```python
from build123d import *

# Parameters (mm, degrees)
CAP_BODY_DEPTH               = 23
BOLT_HOLES_12_D              = 12
SKETCH7_W                    = 17
SKETCH7_H                    = 36
HOLE_34_AT_2_COUNT           = 2
HOLE_34_AT_2_PITCH           = 78
LUBE_COUNTERBORE_SKETCH_8_R  = 4
LUBE_COUNTERBORE_8_DEPTH     = 16
LUBE_HOLE_SKETCH_6_R         = 3
LUBE_HOLE_6_DEPTH            = 72.028163461
SIDE_RELIEF_SKETCH_OUTSIDE_W = 134.804
SIDE_RELIEF_SKETCH_OUTSIDE_H = 72.804
SIDE_RELIEF_CUT_DEPTH        = 66.03076203


with BuildPart() as part:
    # Cap Profile Sketch → Cap Body (new, symmetric)
    with BuildSketch(Plane.XY):
        with BuildLine():
            Line((-22.627416998, 8), (-27.627416998, 8))
            Line((-27.627416998, 8), (-27.627416998, 24))
            Line((-27.627416998, 24), (-54, 24))
            Line((-54, 24), (-54, 36))
            Line((-54, 36), (-31.749015733, 36))
            ThreePointArc((-31.749015733, 36), (0, 48), (31.749015733, 36))
            Line((31.749015733, 36), (54, 36))
            Line((54, 36), (54, 24))
            Line((54, 24), (27.627416998, 24))
            Line((27.627416998, 24), (27.627416998, 8))
            Line((27.627416998, 8), (22.627416998, 8))
            ThreePointArc((22.627416998, 8), (0, 24), (-22.627416998, 8))
        make_face()
    extrude(amount=CAP_BODY_DEPTH, both=True)

    # Bolt Holes Ø12 (through all)
    with Locations(Plane(origin=(0, 36, 0), x_dir=(1, 0, 0), z_dir=(0, 1, 0))):
        with Locations((-39, 0), (39, 0)):
            Hole(BOLT_HOLES_12_D / 2)

    # Sketch7 → Hole Ø34 (revolve, cut)
    with BuildSketch(Plane(origin=(-39, 36, 0), x_dir=(0, 0, -1), z_dir=(1, 0, 0))):
        with Locations((8.5, 18)):
            Rectangle(SKETCH7_W, SKETCH7_H)
    hole_34 = revolve(axis=Axis((-39, 29.65, 0), (0, 1, 0)), mode=Mode.SUBTRACT)

    # Hole Ø34 at 2: Hole Ø34 ×2
    with Locations(*[(i * HOLE_34_AT_2_PITCH, 0, 0) for i in range(1, HOLE_34_AT_2_COUNT)]):
        add(hole_34, mode=Mode.SUBTRACT)

    # Lube Counterbore Sketch Ø8 → Lube Counterbore Ø8 (cut)
    with BuildSketch(Plane(origin=(0, 48, 0), x_dir=(1, 0, 0), z_dir=(0, 1, 0))):
        with Locations(Location((0, 0, 0), (0, 0, 270))):
            Circle(LUBE_COUNTERBORE_SKETCH_8_R)
    extrude(amount=-LUBE_COUNTERBORE_8_DEPTH, mode=Mode.SUBTRACT)

    # Lube Hole Sketch Ø6 → Lube Hole Ø6 (cut, through all)
    with BuildSketch(Plane(origin=(0, 48, 0), x_dir=(1, 0, 0), z_dir=(0, 1, 0))):
        with Locations(Location((0, 0, 0), (0, 0, 270))):
            Circle(LUBE_HOLE_SKETCH_6_R)
    extrude(amount=-LUBE_HOLE_6_DEPTH, mode=Mode.SUBTRACT)

    # Side Relief Sketch outside → Side Relief Cut (cut, through all)
    with BuildSketch(Plane(origin=(0, 36, 0), x_dir=(1, 0, 0), z_dir=(0, 1, 0))):
        Rectangle(SIDE_RELIEF_SKETCH_OUTSIDE_W, SIDE_RELIEF_SKETCH_OUTSIDE_H)
        with BuildLine():
            Line((-31.749015733, 23), (31.749015733, 23))
            Line((31.749015733, 23), (48.856934001, 23))
            ThreePointArc((48.856934001, 23), (54, 0), (48.856934001, -23))
            Line((48.856934001, -23), (31.749015733, -23))
            Line((31.749015733, -23), (-31.749015733, -23))
            Line((-31.749015733, -23), (-48.856934001, -23))
            ThreePointArc((-48.856934001, -23), (-54, 0), (-48.856934001, 23))
            Line((-48.856934001, 23), (-31.749015733, 23))
        make_face(mode=Mode.SUBTRACT)
    extrude(amount=-SIDE_RELIEF_CUT_DEPTH, mode=Mode.SUBTRACT)


solid = part.part
```
Could you check a few things on this model? Use its own coordinates, in mm. A direction names the side the tool comes from. Coordinates: 2 decimals unless noted, no trailing zeros. Order: outer loops, then holes, each group sorted by start corner. A loop starts at its lowest first (then second) coordinate and runs counter-clockwise, first axis right, second up. Notation, with made-up numbers: M -9.75,-24.75 L 8.25,-24.75 A14 cw 8.25,-3.75 Z; hole C 67,81.25 d10. An arc over 180 degrees is marked long. Use a Markdown table: item, result. Add a question column.
Q1. Which directions (+Z, -Z, +X, -X, +Y, -Y) give clear straight access to the entire face, cutting with the end or side of a thin tool? Please do faces 1 (the cylindrical face through (-3.905, 40.112, -0.867)), 2 (the flat face through (-45.3, 36, 0.3)), 3 (the flat face through (27.627, 16, 0)), 4 (the flat face through (34, 36, 5)).
Q2. I want a section at D-D on x = 39. List the corners of the cut face in (y, z) for me.
Q3. I want a section at C-C on z = 0. Give the number of separate pieces and of enclosed holes in the cut face, then the cut area to 3 significant figures.
Q4. We'd pull the mould along X, two halves only. Please class faces 5 (the cylindrical face through (22, 39, 0)), 6 (the flat face through (1, 33, 23)), 7 (the flat face through (3, 32, 1)), 8 (the flat face through (-27.627, 16, 0)): pulls with the +X half, pulls with the -X half, needs draft (parallel to the pull), parting line crosses it, or undercut.
Q5. I want a section at A-A on x = 0. List the corners of the cut face in (y, z) for me.
Q6. I want a section at B-B on y = 31. List the corners of the cut face in (x, z) for me, then the cut area to 3 significant figures.
Q7. I'm going to push flat-ended pins straight in: pin 1 (2 mm diameter, centred on x = 36, y = 36.5, fed in from +Z); pin 2 (1 mm diameter, centred on x = -40, z = 7, fed in from +Y); pin 3 (8 mm diameter, centred on x = 15, z = -6, fed in from +Y); pin 4 (13 mm diameter, centred on x = 38, z = 0.5, fed in from -Y). Where does each tip first touch, or does it pass through?
Q8. If I drill on L1, parallel to Z at x = 0, y = 29; L2, parallel to Z at x = 39, y = 30.75; L3, parallel to Y at x = 24, z = 1.5, over which ranges is the centre line in solid material (lowest first)?
Checked values:
| question | item | result |
|---|---|---|
| 1 | face 1 | +Y |
| 1 | face 2 | -X, +Y |
| 1 | face 3 | +Z, -Z, +X, -Y |
| 1 | face 4 | +X, +Y |
| 2 | outline | M 24,-23 L 36,-23 L 36,-6 L 24,-6 Z; M 24,6 L 36,6 L 36,23 L 24,23 Z |
| 3 | separate pieces | 4 |
| 3 | enclosed holes | 0 |
| 3 | area | 1,640 mm² |
| 4 | face 5 | pulls with the +X half |
| 4 | face 6 | needs draft |
| 4 | face 7 | undercut |
| 4 | face 8 | pulls with the -X half |
| 5 | outline | M 24,-23 L 48,-23 L 48,-4 L 32,-4 L 32,-3 L 24,-3 Z; M 24,3 L 32,3 L 32,4 L 48,4 L 48,23 L 24,23 Z |
| 6 | outline | M -48.86,-23 L 48.86,-23 A54 ccw 48.86,23 L -48.86,23 A54 ccw Z; hole C -39,0 d12; hole C 0,0 d6; hole C 39,0 d12 |
| 6 | area | 4,560 mm² |
| 7 | pin 1 | z = 23 |
| 7 | pin 2 | y = 36 |
| 7 | pin 3 | y = 46.72 |
| 7 | pin 4 | y = 24 |
| 8 | L1 | -23 to -3, 3 to 23 |
| 8 | L2 | -23 to -6, 6 to 23 |
| 8 | L3 | 8 to 36 |
